```python
from build123d import *

# Parameters (mm, degrees)
SKETCH_1_W                  = 65
SKETCH_1_H                  = 25
SKETCH_1_R                  = 1.6
EXTRUDE_1_DEPTH             = 3
FILLET_1_R                  = 2
HOLE_WIZARD_4_3_4_3_1_D     = 4.3
HOLE_WIZARD_4_3_4_3_1_DEPTH = 11.5
HOLE_WIZARD_4_3_4_3_1_TIP   = 1.291850331
SKETCH_4_W                  = 10
SKETCH_4_H                  = 22
EXTRUDE_2_DEPTH             = 3
SKETCH_5_R                  = 2.1
CUT_EXTRUDE_1_DEPTH         = 10
FILLET_2_R                  = 2
HOLE_WIZARD_M3_1_D          = 2.5
HOLE_WIZARD_M3_1_DEPTH      = 8.5
HOLE_WIZARD_M3_1_TIP        = 0.751075774


with BuildPart() as part:
    # 草图1 → 凸台-拉伸1 (new body)
    with BuildSketch(Plane(origin=(0, 0, 0), x_dir=(0, 0, -1), z_dir=(1, 0, 0))):
        Rectangle(SKETCH_1_W, SKETCH_1_H)
        with Locations((-26.5, 7.5)):
            Circle(SKETCH_1_R, mode=Mode.SUBTRACT)
        with Locations(Location((-26.5, -7.5, 0), (0, 0, 180))):
            Circle(SKETCH_1_R, mode=Mode.SUBTRACT)
    extrude(amount=EXTRUDE_1_DEPTH)

    # 圆角1
    fillet_1_edges = [part.edges().sort_by_distance(p)[0] for p in [
        (1.5, -12.5, -32.5),
        (1.5, -12.5, 32.5),
        (1.5, 12.5, 32.5),
        (1.5, 12.5, -32.5),
    ]]
    fillet(fillet_1_edges, radius=FILLET_1_R)

    # Ø4.3 (4.3) 直径孔1
    with Locations(Plane.ZY):
        with Locations((-27.5, 8), (-27.5, -8), (-27.5, 0)):
            Hole(HOLE_WIZARD_4_3_4_3_1_D / 2, depth=HOLE_WIZARD_4_3_4_3_1_DEPTH)
            with Locations((0, 0, -(HOLE_WIZARD_4_3_4_3_1_DEPTH + HOLE_WIZARD_4_3_4_3_1_TIP / 2))):  # 118° drill point
                Cone(0, HOLE_WIZARD_4_3_4_3_1_D / 2, HOLE_WIZARD_4_3_4_3_1_TIP, mode=Mode.SUBTRACT)

    # 草图4 → 凸台-拉伸2 (add)
    with BuildSketch(Plane(origin=(3, 0, 0), x_dir=(0, 0, -1), z_dir=(1, 0, 0))):
        with Locations((-12.5, 12.5)):
            Rectangle(SKETCH_4_W, SKETCH_4_H)
    extrude(amount=-EXTRUDE_2_DEPTH)

    # 草图5 → 切除-拉伸1 (cut)
    with BuildSketch(Plane.ZY):
        with Locations((12.5, 20.6)):
            Circle(SKETCH_5_R)
    extrude(amount=-CUT_EXTRUDE_1_DEPTH, mode=Mode.SUBTRACT)

    # 圆角2
    fillet_2_edges = [part.edges().sort_by_distance(p)[0] for p in [
        (1.5, 12.5, 17.5),
        (1.5, 12.5, 7.5),
        (1.5, 23.5, 7.5),
        (1.5, 23.5, 17.5),
    ]]
    fillet(fillet_2_edges, radius=FILLET_2_R)

    # M3 螺纹孔1
    with Locations(Plane.ZY):
        with Locations((12.5, 6.6), (12.5, 13.1)):
            Hole(HOLE_WIZARD_M3_1_D / 2, depth=HOLE_WIZARD_M3_1_DEPTH)
            with Locations((0, 0, -(HOLE_WIZARD_M3_1_DEPTH + HOLE_WIZARD_M3_1_TIP / 2))):  # 118° drill point
                Cone(0, HOLE_WIZARD_M3_1_D / 2, HOLE_WIZARD_M3_1_TIP, mode=Mode.SUBTRACT)


solid = part.part
```
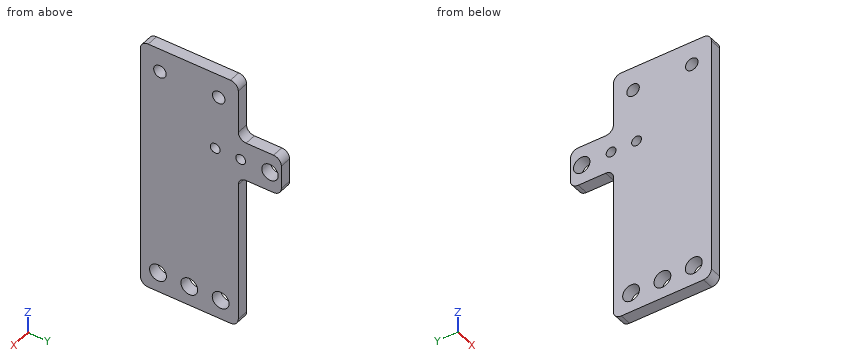
The listing builds one solid part. Answer for the finished solid, in the listing's coordinates (mm). Give positions to 0.01 mm unless a question says otherwise; leave off trailing zeros. Order: outer loops, then holes, each group sorted by start corner. A loop starts at its lowest first (then second) coordinate and runs counter-clockwise, first axis right, second up. Notation, with made-up numbers: (49.5, -19.5) -> (88.5, -19.5) arc R29 ccw to (88.5, 15.5) -> close; hole circle Ø7 at (88.5, -22.75). An arc over 180 degrees is marked (long way). Answer as CSV lines item,"result". Start each with the question number.
Q1. A cutting plane is placed at A-A (z = -26.5). Determine the outline of the cut face in (x, y), then the cut area to 3 significant figures.
Q2. A cutting plane is placed at C-C (z = 27.5). Determine the outline of the cut face in (x, y), then the cut area to 3 significant figures.
Q3. Given pin 1 (7 mm diameter, centred on y = 0, z = -27.5, fed in from -X), flat-ended and moving along its own axis, determine where the tip first touches the part or whether it passes through.
Q4. Find the intervals of material crossed by L1, parallel to Y at x = 1.7, z = -27.5; L2, parallel to Y at x = 1.4, z = 26.5; L3, parallel to Z at x = 2.5, y = 7, in increasing order.
Q5. A cutting plane is placed at D-D (z = -14). Determine the outline of the cut face in (x, y), then the cut area to 3 significant figures.
Q6. A cutting plane is placed at B-B (x = 0.95). Count the separate pieces of the cut face and the enclosed holes in it, then the cut area to 3 significant figures.
Results found:
1,outline,"(0, -12.5) -> (3, -12.5) -> (3, -9.9) -> (0, -9.9) -> close; (0, -6.1) -> (3, -6.1) -> (3, -1.9) -> (0, -1.9) -> close; (0, 1.9) -> (3, 1.9) -> (3, 6.1) -> (0, 6.1) -> close; (0, 9.9) -> (3, 9.9) -> (3, 12.5) -> (0, 12.5) -> close"
1,area,"40.7 mm2"
2,outline,"(0, -12.5) -> (3, -12.5) -> (3, -8.75) -> (0, -8.75) -> close; (0, -6.25) -> (3, -6.25) -> (3, 6.25) -> (0, 6.25) -> close; (0, 8.75) -> (3, 8.75) -> (3, 12.5) -> (0, 12.5) -> close"
2,area,"60.0 mm2"
3,pin 1,"x = 0"
4,L1,"-12.5 to -10.15, -5.85 to -2.15, 2.15 to 5.85, 10.15 to 12.5"
4,L2,"-12.5 to -9.1, -5.9 to 5.9, 9.1 to 12.5"
4,L3,"-32.5 to -29.4, -25.6 to 11.32, 13.68 to 24.98, 28.02 to 32.5"
5,outline,"(0, -12.5) -> (3, -12.5) -> (3, 12.5) -> (0, 12.5) -> close"
5,area,"75.0 mm2"
6,separate pieces,"1"
6,enclosed holes,"8"
6,area,"1,650 mm2"
